```python
from build123d import *

# Parameters (mm, degrees)
STEP_PLATE_10MM_DEPTH = 5
DRAFT_15DEG_ANGLE     = -15


with BuildPart() as part:
    # Step Plate Profile → Step Plate 10mm (new, symmetric)
    with BuildSketch(Plane(origin=(0, 0, 0), x_dir=(0, 0, -1), z_dir=(1, 0, 0))):
        Polygon((0, 0), (170, 0), (170, 50), (160, 50), (160, 20), (150, 20), (150, 50), (20, 50), (20, 20), (10, 20), (10, 50), (0, 50), align=None)
    extrude(amount=STEP_PLATE_10MM_DEPTH, both=True)

    # Draft 15deg
    draft_15deg_faces = [part.faces().sort_by_distance(p)[0] for p in [
        (0, 0, -85),
    ]]
    draft(draft_15deg_faces, Plane(origin=(-5, 0, 0), x_dir=(0, 0, -1), z_dir=(-1, 0, 0)), DRAFT_15DEG_ANGLE)


solid = part.part
```
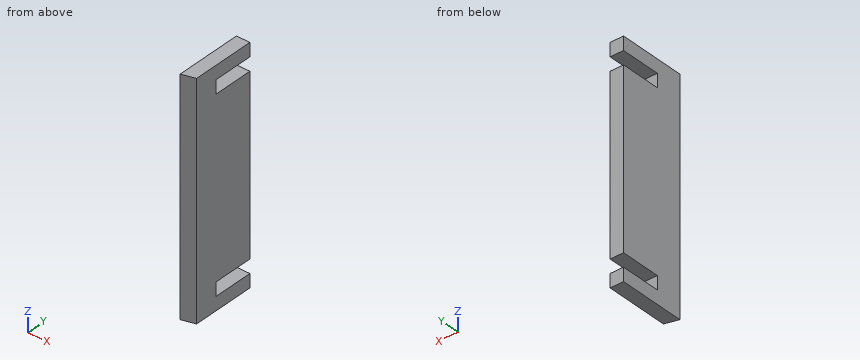
Geometry: final body of the model. Coordinates: model frame, mm. Give positions to 0.01 mm unless a question says otherwise; leave off trailing zeros. Write each loop counter-clockwise with the first axis right and the second up, starting at its lowest first coordinate (ties: lowest second). Pieces come first, ordered by that corner, then holes.
1. Section query B-B, the plane x = -2.25. Return loops of the section in (y, z).
2. Line query: probe 1 along Z at (x, y) = (-0.5, 39); probe 2 along Y at (x, z) = (-4.25, -158); probe 3 along Y at (x, z) = (-0.5, -16.5). Output: solid intervals per line, ascending.
3. Section query A-A, the plane y = 39. Return loops of the section in (x, z).
4. Section query C-C, the plane z = -138. Return loops of the section in (x, y), then the cut area to 3 significant figures.
5. Pin query (flat end, axial travel): P1, Ø2, axis at x = -3.5, z = -53, coming from the -Y side; P2, Ø1.5, axis at x = 3.5, z = -45.5, coming from the -Y side; P3, Ø5, axis at x = -1.5, z = -157, coming from the +Y side. Return the tip coordinate at first contact, or that it passes through.
Computed:
1. outline: (0.74, -170) - (50, -170) - (50, -160) - (20, -160) - (20, -150) - (50, -150) - (50, -20) - (20, -20) - (20, -10) - (50, -10) - (50, 0) - (0.74, 0) - close
2. probe 1: z = -170 to -160, -150 to -20, -10 to 0
2. probe 2: y = 0.2 to 20
2. probe 3: y = 1.21 to 20
3. outline: (-5, -170) - (5, -170) - (5, -160) - (-5, -160) - close; (-5, -150) - (5, -150) - (5, -20) - (-5, -20) - close; (-5, -10) - (5, -10) - (5, 0) - (-5, 0) - close
4. outline: (-5, 0) - (5, 2.68) - (5, 50) - (-5, 50) - close
4. area: 487 mm2
5. P1: stops at y = 0.13
5. P2: stops at y = 2.08
5. P3: stops at y = 20
